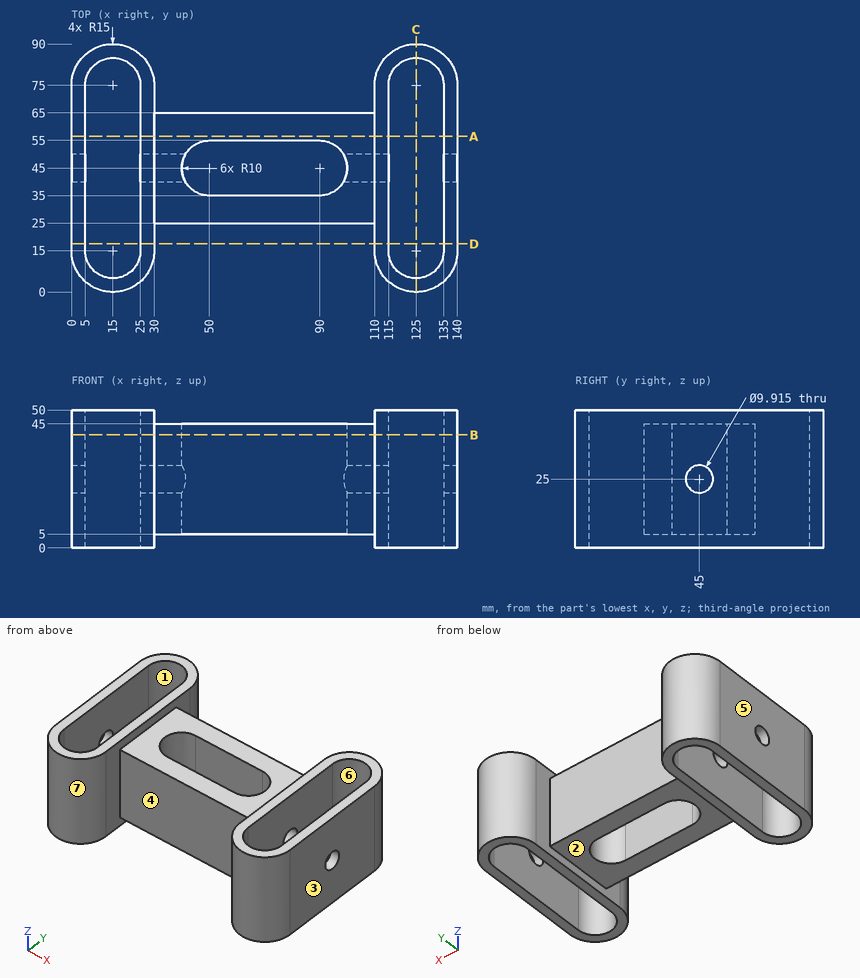
Input: dimensioned drawing with shaded views. Units: mm. Origin: part minimum x, y, z. A direction names the side the tool comes from. Give positions to 0.01 mm unless a question says otherwise; leave off trailing zeros. Write each loop counter-clockwise with the first axis right and the second up, starting at its lowest first coordinate (ties: lowest second). Pieces come first, ordered by that corner, then holes. Notation, with made-up numbers: (2.5, 35) -> (14.5, 35) arc R33 ccw to (14.5, 65) -> close; hole circle Ø2 at (-10.5, 39.5). An arc over 180 degrees is marked (long way). Answer as a JSON object with one key per item and string values.
1. Cut plane B-B on z = 41. Output: boundary loops of the cut face in (x, y).
Ans:
{"outline": "(0, 15) arc R15 ccw to (30, 15) -> (30, 25) -> (110, 25) -> (110, 15) arc R15 ccw to (140, 15) -> (140, 75) arc R15 ccw to (110, 75) -> (110, 65) -> (30, 65) -> (30, 75) arc R15 ccw to (0, 75) -> close; hole (5, 15) arc R10 ccw to (25, 15) -> (25, 75) arc R10 ccw to (5, 75) -> close; hole (50, 35) -> (90, 35) arc R10 ccw to (90, 55) -> (50, 55) arc R10 ccw to start; hole (115, 15) arc R10 ccw to (135, 15) -> (135, 75) arc R10 ccw to (115, 75) -> close"}
2. Ray query, probe 1 along X at (y, z) = (67, 23.5); probe 2 along X at (y, z) = (45.5, 12); probe 3 along Y at (x, z) = (31.5, 25). Return the intervals inside material, ascending. Write a range as from..to.
Ans:
{"probe 1": "x = 0..5, 25..30, 110..115, 135..140", "probe 2": "x = 0..5, 25..40.01, 99.99..115, 135..140", "probe 3": "y = 25..40.04, 49.96..65"}
3. Access query for the marked faces 1, 2, 3 and 4. Directions: +Z, -Z, +X, -X, +Y, -Y. A direction counts if a zero-diameter tool reaches every point of the face in a straight line with its end or side. Return the directions, or none.
Ans:
{"face 1": "+Z, -Z", "face 2": "-Z, +Y, -Y", "face 3": "+Z, -Z, +X, +Y, -Y", "face 4": "+Z, -Z, -Y"}
4. Cut plane D-D on y = 17.5. Output: boundary loops of the cut face in (x, z), and give its area (3 significant figures).
Ans:
{"outline": "(0, 0) -> (5, 0) -> (5, 50) -> (0, 50) -> close; (25, 0) -> (30, 0) -> (30, 50) -> (25, 50) -> close; (110, 0) -> (115, 0) -> (115, 50) -> (110, 50) -> close; (135, 0) -> (140, 0) -> (140, 50) -> (135, 50) -> close", "area": "1,000 mm^2"}
5. Cut plane A-A on y = 56.5. Output: boundary loops of the cut face in (x, z).
Ans:
{"outline": "(0, 0) -> (5, 0) -> (5, 50) -> (0, 50) -> close; (25, 0) -> (30, 0) -> (30, 5) -> (110, 5) -> (110, 0) -> (115, 0) -> (115, 50) -> (110, 50) -> (110, 45) -> (30, 45) -> (30, 50) -> (25, 50) -> close; (135, 0) -> (140, 0) -> (140, 50) -> (135, 50) -> close"}
6. Contact query for flat-ended pins moving along their axis: pin 1 (6 mm diameter, centred on y = 45, z = 25, fed in from -X); pin 2 (12 mm diameter, centred on x = 73, z = 19.5, fed in from +Y); pin 3 (20 mm diameter, centred on x = 80, y = 49, fed in from -Z); pin 4 (20 mm diameter, centred on x = 66.5, z = 22.5, fed in from -Y). Output: stop coordinate, or through.
Ans:
{"pin 1": "passes through", "pin 2": "stops at y = 65", "pin 3": "stops at z = 5", "pin 4": "stops at y = 25"}
7. Mould query, pull axis Y, two halves, no side actions, for the marked faces 5, 6 and 7. Classes: pulls with the +Y half, pulls with the -Y half, needs draft (parallel to the pull), parting line crosses it, or undercut.
Ans:
{"face 5": "needs draft", "face 6": "undercut", "face 7": "pulls with the -Y half"}
8. Cut plane C-C on x = 125. Output: boundary loops of the cut face in (y, z), and give its area (3 significant figures).
Ans:
{"outline": "(0, 0) -> (5, 0) -> (5, 50) -> (0, 50) -> close; (85, 0) -> (90, 0) -> (90, 50) -> (85, 50) -> close", "area": "500 mm^2"}
